Could you check a few things on this model? Use its own coordinates, in mm. A direction names the side the tool comes from. Coordinates: 2 decimals unless noted, no trailing zeros. Loops run counter-clockwise (first coordinate to the right, second up) from the corner with the lowest first, then second, coordinate; pieces in that order, holes last.
from build123d import *

# Parameters (mm, degrees)
SKETCH1_W                                           = 150
SKETCH1_H                                           = 25
BOSS_EXTRUDE1_DEPTH                                 = 12
CBORE_FOR_M5_HEX_SOCKET_HEAD_CAP_SCREW1_D           = 5.5
CBORE_FOR_M5_HEX_SOCKET_HEAD_CAP_SCREW1_CBORE_D     = 10
CBORE_FOR_M5_HEX_SOCKET_HEAD_CAP_SCREW1_CBORE_DEPTH = 5
CHAMFER1_SIZE                                       = 0.5


with BuildPart() as part:
    # Sketch1 → Boss-Extrude1 (new body)
    with BuildSketch(Plane.XY):
        Rectangle(SKETCH1_W, SKETCH1_H)
    extrude(amount=BOSS_EXTRUDE1_DEPTH)

    # CBORE for M5 Hex Socket Head Cap Screw1 (through all)
    with Locations(Plane.XY.offset(12)):
        with Locations((0, -5), (-65, -5), (65, -5)):
            CounterBoreHole(CBORE_FOR_M5_HEX_SOCKET_HEAD_CAP_SCREW1_D / 2, CBORE_FOR_M5_HEX_SOCKET_HEAD_CAP_SCREW1_CBORE_D / 2, CBORE_FOR_M5_HEX_SOCKET_HEAD_CAP_SCREW1_CBORE_DEPTH)

    # Chamfer1
    chamfer1_edges = [part.edges().sort_by_distance(p)[0] for p in [
        (75, -12.5, 6),
        (-75, -12.5, 6),
        (-75, 12.5, 6),
        (75, 12.5, 6),
    ]]
    chamfer(chamfer1_edges, length=CHAMFER1_SIZE)


solid = part.part
(1) I need wall thicknesses on probe 1 along Y at (x, z) = (0, 2.5); probe 2 along Y at (x, z) = (-65, 11); probe 3 along X at (y, z) = (-3.25, 10.5). Which ranges of each line are inside material? Lowest first, please.
Answers:
probe 1: y = -12.5 to -7.75, -2.25 to 12.5
probe 2: y = -12.5 to -10, 0 to 12.5
probe 3: x = -75 to -69.68, -60.32 to -4.68, 4.68 to 60.32, 69.68 to 75
(2) Imagine slicing it at C-C, the plane z = 2.25. Write out the boundary of the cut face in (x, y), and give its area (3 significant figures).
Answers:
outline: (-75, -12) - (-74.5, -12.5) - (74.5, -12.5) - (75, -12) - (75, 12) - (74.5, 12.5) - (-74.5, 12.5) - (-75, 12) - close; hole circle Ø5.5 at (-65, -5); hole circle Ø5.5 at (0, -5); hole circle Ø5.5 at (65, -5)
area: 3,680 mm2
(3) Which directions (+Z, -Z, +X, -X, +Y, -Y) give clear straight access to the entire face, cutting with the end or side of a thin tool? Please do faces 1 (the face through (-1, 12.5, 6)), 2 (the face through (67.2, -7.2, 7)).
Answers:
face 1: +Z, -Z, +X, -X, +Y
face 2: +Z
(4) Imagine slicing it at A-A, the plane y = -5. Write out the boundary of the cut face in (x, z).
Answers:
outline: (-75, 0) - (-67.75, 0) - (-67.75, 7) - (-70, 7) - (-70, 12) - (-75, 12) - close; (-62.25, 0) - (-2.75, 0) - (-2.75, 7) - (-5, 7) - (-5, 12) - (-60, 12) - (-60, 7) - (-62.25, 7) - close; (2.75, 0) - (62.25, 0) - (62.25, 7) - (60, 7) - (60, 12) - (5, 12) - (5, 7) - (2.75, 7) - close; (67.75, 0) - (75, 0) - (75, 12) - (70, 12) - (70, 7) - (67.75, 7) - close
(5) We'd pull the mould along X, two halves only. Please class faces 3 (the face through (0.596, -7.685, 3.451)), 4 (the face through (-70, -5, 10)), 5 (the face through (-1, 0, 0)), 6 (the face through (75, 0, 6)): +X half, -X half, draft (parallel to the pull), parting line (faces both ways), or undercut.
Answers:
face 3: undercut
face 4: undercut
face 5: draft
face 6: +X half
(6) Imagine slicing it at B-B, the plane x = 0. Write out the boundary of the cut face in (y, z).
Answers:
outline: (-12.5, 0) - (-7.75, 0) - (-7.75, 7) - (-10, 7) - (-10, 12) - (-12.5, 12) - close; (-2.25, 0) - (12.5, 0) - (12.5, 12) - (0, 12) - (0, 7) - (-2.25, 7) - close
(7) For pin 1 (8 mm diameter, centred on x = 65, y = -5, fed in from +Z); pin 2 (4.5 mm diameter, centred on x = 65, y = -5, fed in from -Z); pin 3 (11 mm diameter, centred on x = 65.5, y = -6.5, fed in from +Z), each with a flat end and sliding along its axis, tell me the tip position at first contact or that it passes through.
Answers:
pin 1: stops at z = 7
pin 2: passes through
pin 3: stops at z = 12
